Geometry: see drawing. Coordinates: mm, zero at the bounding-box minimum. A direction names the side the tool comes from. Round coordinates to 2 decimals unless told otherwise and drop trailing zeros. Loops run counter-clockwise (first coordinate to the right, second up) from the corner with the lowest first, then second, coordinate; pieces in that order, holes last. Notation, with made-up numbers: (-16, -25) - (20, -25) arc R19 ccw to (20, -19) - close; hole circle Ø7 at (-10, 22.5). An arc over 180 degrees is marked (long way). Use CSV: the item, a comma, the result in double quotes. Start each with the question number.
1. Cut plane B-B (y = 97). Return loops of the section in (x, z).
2. Access query for the marked faces 1, 2, 3 and 4. Directions: +Z, -Z, +X, -X, +Y, -Y. A direction counts if a zero-diameter tool reaches every point of the face in a straight line with its end or side. Return the directions, or none.
3. Cut plane D-D (z = 45.5). Return loops of the section in (x, y) (1 decimal).
4. Cut plane A-A (x = 100). Return loops of the section in (y, z), and give its area (3 significant figures).
5. Pin query (flat end, axial travel): P1, Ø5, axis at x = 143, y = 15.5, coming from the -Z side; P2, Ø6, axis at y = 70, z = 37.5, coming from the +X side; P3, Ø8, axis at x = 44.5, z = 13, coming from the +Y side; P4, Ø6, axis at x = 190, z = 10, coming from the +Y side. Return the tip coordinate at first contact, or that it passes through.
6. Cut plane C-C (x = 133.5). Return loops of the section in (y, z).
7. Material intervals for probe 1 along Z at (x, y) = (190, 5.25); probe 2 along Z at (x, y) = (112.5, 90); probe 3 along X at (y, z) = (168, 78), sorted ascending. Write a range as from..to.
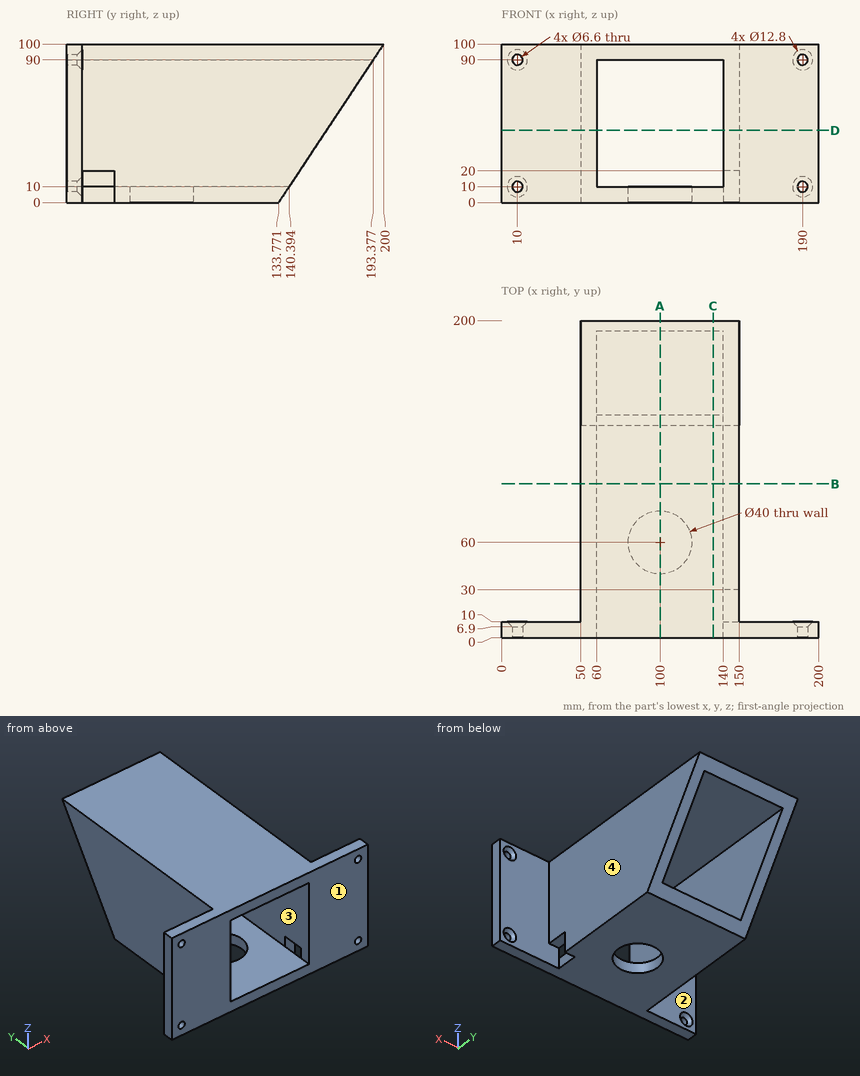
Established:
1,outline,"(50, 0) - (150, 0) - (150, 100) - (50, 100) - close; hole (60, 10) - (140, 10) - (140, 90) - (60, 90) - close"
2,face 1,"+Z, -Z, +X, -X, -Y"
2,face 2,"+Z, -Z, -X, +Y"
2,face 3,"+Y, -Y"
2,face 4,"+Z, -Z, +X, +Y"
3,outline,"(0, 0) - (60, 0) - (60, 163.9) - (50, 163.9) - (50, 10) - (0, 10) - close; (140, 0) - (200, 0) - (200, 10) - (150, 10) - (150, 163.9) - (140, 163.9) - close"
4,outline,"(0, 0) - (40, 0) - (40, 10) - (0, 10) - close; (0, 90) - (193.38, 90) - (200, 100) - (0, 100) - close; (80, 0) - (133.77, 0) - (140.39, 10) - (80, 10) - close"
4,area,"2,940 mm2"
5,P1,"stops at z = 20"
5,P2,"stops at x = 150"
5,P3,"stops at y = 10"
5,P4,"passes through"
6,outline,"(0, 0) - (133.77, 0) - (140.39, 10) - (0, 10) - close; (0, 90) - (193.38, 90) - (200, 100) - (0, 100) - close"
7,probe 1,"z = 0..6.7, 13.3..86.7, 93.3..100"
7,probe 2,"z = 0..10, 90..100"
7,probe 3,"x = 50..60, 140..150"
